from build123d import *

# Parameters (mm, degrees)
EXTRUDE_1_DEPTH     = 875
SKETCH_2_W          = 100
SKETCH_2_H          = 60
CUT_EXTRUDE_2_DEPTH = 1017.542118193


with BuildPart() as part:
    # 草图1 → 凸台-拉伸1 (new, symmetric)
    with BuildSketch(Plane.XY):
        Polygon((-295.14043786, 27.019055308), (-295.14043786, 2.019055308), (114.859562138, 2.019055308), (114.859562138, 425), (89.859562138, 425), (89.859562138, 27.019055308), align=None)
    extrude(amount=EXTRUDE_1_DEPTH, both=True)

    # 草图2 → 切除-拉伸2 (cut, through all)
    with BuildSketch(Plane(origin=(0, 0, 0), x_dir=(0, 0, -1), z_dir=(1, 0, 0))):
        with Locations((725, 330)):
            Rectangle(SKETCH_2_W, SKETCH_2_H)
        with Locations((-745, 330)):
            Rectangle(SKETCH_2_W, SKETCH_2_H)
        with Locations((725, 122.019055308)):
            Rectangle(SKETCH_2_W, SKETCH_2_H)
        with Locations((-745, 122.019055308)):
            Rectangle(SKETCH_2_W, SKETCH_2_H)
    extrude(amount=CUT_EXTRUDE_2_DEPTH, mode=Mode.SUBTRACT)


solid = part.part
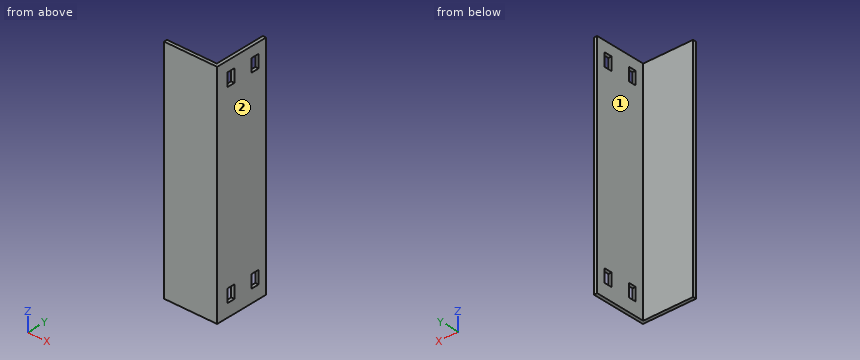
Could you check a few things on this model? Use its own coordinates, in mm. Face numbers are marked on the shaded views. A direction names the side the tool comes from. Round coordinates to 2 decimals unless told otherwise and drop trailing zeros. Write each loop counter-clockwise with the first axis right and the second up, starting at its lowest first coordinate (ties: lowest second). Pieces come first, ordered by that corner, then holes. Notation, with made-up numbers: (-1.5, -36) - (48.5, -36) arc R29 cw to (48.5, -1) - close; hole circle Ø2 at (-21.5, 18.5). An arc over 180 degrees is marked (long way). Put each result on its own line as item: value. Start each with the question number.
(1) I want a section at D-D, the plane y = 215.5. Please give me the cut outline in (x, z).
(2) I want a section at A-A, the plane z = 766.5. Please give me the cut outline in (x, y).
(3) Will these pins go through, and if not, where does the flat tip stop? pin 1 (3 mm diameter, centred on y = 268, z = 614.5, fed in from -X); pin 2 (3 mm diameter, centred on x = -199, z = -492.5, fed in from +Y).
(4) I want a section at B-B, the plane y = 112.5. Please give me the cut outline in (x, z).
(5) For the marked faces 1 and 2, which set-ups out of +Z, -Z, +X, -X, +Y, -Y let a thin tool reach every point of the face, with its end or its side?
(6) I want a section at C-C, the plane z = -47.5. Please give me the cut outline in (x, y).
(7) I need wall thicknesses on probe 1 along Y at (x, z) = (4.5, -586.5); probe 2 along X at (y, z) = (82, -316.5). Which ranges of each line are inside material? Lowest first, please.
Here are the results:
1. outline: (89.86, -875) - (114.86, -875) - (114.86, 875) - (89.86, 875) - close
2. outline: (-295.14, 2.02) - (114.86, 2.02) - (114.86, 92.02) - (89.86, 92.02) - (89.86, 27.02) - (-295.14, 27.02) - close; (89.86, 152.02) - (114.86, 152.02) - (114.86, 300) - (89.86, 300) - close; (89.86, 360) - (114.86, 360) - (114.86, 425) - (89.86, 425) - close
3. pin 1: stops at x = 89.86
3. pin 2: stops at y = 27.02
4. outline: (89.86, -875) - (114.86, -875) - (114.86, -775) - (89.86, -775) - close; (89.86, -675) - (114.86, -675) - (114.86, 695) - (89.86, 695) - close; (89.86, 795) - (114.86, 795) - (114.86, 875) - (89.86, 875) - close
5. face 1: +Z, -Z, -X, +Y
5. face 2: +Z, -Z, +X, +Y, -Y
6. outline: (-295.14, 2.02) - (114.86, 2.02) - (114.86, 425) - (89.86, 425) - (89.86, 27.02) - (-295.14, 27.02) - close
7. probe 1: y = 2.02 to 27.02
7. probe 2: x = 89.86 to 114.86
